Build history of the part. All positions in model axes, mm. A direction names the side the tool comes from. Round coordinates to 2 decimals unless told otherwise and drop trailing zeros. Write each loop counter-clockwise with the first axis right and the second up, starting at its lowest first coordinate (ties: lowest second). Pieces come first, ordered by that corner, then holes. Notation, with made-up numbers: (73, 52.5) -> (84, 52.5) arc R29 ccw to (84, 73.5) -> close; hole circle Ø2 at (27, -10.5). An arc over 180 degrees is marked (long way). One line per question, with ' | ' between items.
from build123d import *

# Parameters (mm, degrees)
BASE_PLATE_SKETCH_W       = 60
BASE_PLATE_SKETCH_H       = 40
BASE_PLATE_60X40X10_DEPTH = 5
UPRIGHT_LUG_SKETCH_W      = 60
UPRIGHT_LUG_SKETCH_H      = 20
UPRIGHT_LUG_DEPTH         = 30
CROSS_HOLE_SKETCH_R       = 10
CROSS_HOLE_CUT_DEPTH      = 62.032778079
LUG_PROFILE_CUT_DEPTH     = 62.032778079
LUG_ROUND_R10_R           = 10


with BuildPart() as part:
    # Base Plate Sketch → Base Plate 60x40x10 (new, symmetric)
    with BuildSketch(Plane(origin=(0, 0, 0), x_dir=(1, 0, 0), z_dir=(0, 1, 0))):
        Rectangle(BASE_PLATE_SKETCH_W, BASE_PLATE_SKETCH_H)
    extrude(amount=BASE_PLATE_60X40X10_DEPTH, both=True)

    # Upright Lug Sketch → Upright Lug (add)
    with BuildSketch(Plane(origin=(0, 5, 0), x_dir=(1, 0, 0), z_dir=(0, 1, 0))):
        with Locations((0, 10)):
            Rectangle(UPRIGHT_LUG_SKETCH_W, UPRIGHT_LUG_SKETCH_H)
    extrude(amount=UPRIGHT_LUG_DEPTH)

    # Cross Hole Sketch → Cross Hole Cut (cut, through all)
    with BuildSketch(Plane(origin=(0, 0, -20), x_dir=(-1, 0, 0), z_dir=(0, 0, -1))):
        with Locations((-10, 15)):
            Circle(CROSS_HOLE_SKETCH_R)
    extrude(amount=-CROSS_HOLE_CUT_DEPTH, mode=Mode.SUBTRACT)

    # Lug Profile Sketch → Lug Profile Cut (cut, through all)
    with BuildSketch(Plane(origin=(0, 0, -20), x_dir=(-1, 0, 0), z_dir=(0, 0, -1))):
        with BuildLine():
            Line((-30, 35), (-30, 15.000000101))
            ThreePointArc((-30, 15.000000101), (-24.142135638, 29.142135609), (-10.000000142, 35))
            Line((-10.000000142, 35), (-30, 35))
        make_face()
        with BuildLine():
            ThreePointArc((-10.000000142, 35), (4.142135574, 29.142135674), (10, 15))
            Line((10, 15), (30, 15))
            Line((30, 15), (30, 35))
            Line((30, 35), (-10.000000142, 35))
        make_face()
    extrude(amount=-LUG_PROFILE_CUT_DEPTH, mode=Mode.SUBTRACT)

    # Lug Round R10
    lug_round_r10_edges = [part.edges().sort_by_distance(p)[0] for p in [
        (-30, 15, -10),
    ]]
    fillet(lug_round_r10_edges, radius=LUG_ROUND_R10_R)


solid = part.part
(1) Slice it at A-A (z = -11). Write the cut outline in (x, y).
Calculated:
outline: (-30, -5) -> (30, -5) -> (30, 15) arc R20 ccw to (-10, 15) -> (-20, 15) arc R10 ccw to (-30, 5) -> close; hole circle Ø20 at (10, 15)
(2) 3-axis set-ups, long thin cutter, end or side, ignore diameter. For faces 5 (the flat face through (0, 5, 10)), 6 (the flat face through (-15, 15, -10)), 7 (the flat face through (0, 10, -20)): which of +Z, -Z, +X, -X, +Y, -Y reach the whole face in a straight line?
Calculated:
face 5: +Z, +X, -X, +Y | face 6: +Z, -Z, -X, +Y | face 7: -Z, +X, -X, +Y, -Y
(3) Slice it at C-C (z = 6). Write the cut outline in (x, y), then the cut area to 3 significant figures.
Calculated:
outline: (-30, -5) -> (30, -5) -> (30, 5) -> (-30, 5) -> close | area: 600 mm2
(4) Wall check: line 1 (Z direction, x = 27.5, y = 12.5); line 2 (Y direction, x = 4.5, z = 12); line 3 (Y direction, x = -14, z = -6). Give the ranges that are in metal, low to high. Write a range as from..to.
Calculated:
line 1: -20..0 | line 2: -5..5 | line 3: -5..15
(5) Drop flat-ended pins along their axis: pin 1 (1 mm diameter, centred on x = -3, y = 6, fed in from +Z); pin 2 (8 mm diameter, centred on x = -16.5, z = -8, fed in from +Y); pin 3 (12 mm diameter, centred on y = 14.5, z = 3, fed in from -X). Give the stop position or say it passes through.
Calculated:
pin 1: z = 0 | pin 2: y = 15 | pin 3: x = -29.03
(6) Mould opens along X. For faces 1 (the flat face through (30, 3, -4)), 2 (the cylindrical face through (-27.15, 11.99, -9.86)), 3 (the cylindrical face through (4.62, 23.43, -10.14)), 4 (the flat face through (0, 0, 20)) say: pulls with the +X half, pulls with the -X half, needs draft (parallel to the pull), parting line crosses it, or undercut.
Calculated:
face 1: pulls with the +X half | face 2: pulls with the -X half | face 3: undercut | face 4: needs draft
(7) Slice it at D-D (x = -3). Write the cut outline in (y, z), then the cut area to 3 significant figures.
Calculated:
outline: (-5, -20) -> (30.2, -20) -> (30.2, 0) -> (5, 0) -> (5, 20) -> (-5, 20) -> close | area: 904 mm2
(8) Slice it at B-B (x = 13.5). Write the cut outline in (y, z).
Calculated:
outline: (-5, -20) -> (5.63, -20) -> (5.63, 0) -> (5, 0) -> (5, 20) -> (-5, 20) -> close; (24.37, -20) -> (34.69, -20) -> (34.69, 0) -> (24.37, 0) -> close
